Could you check a few things on this model? Use its own coordinates, in mm. Coordinates: 2 decimals unless noted, no trailing zeros. Loops run counter-clockwise (first coordinate to the right, second up) from the corner with the lowest first, then second, coordinate; pieces in that order, holes last. Notation, with made-up numbers: M 80,48.5 L 131,48.5 A16 cw 131,64.5 Z; hole C -8.5,66 d9. An arc over 180 degrees is marked long. Use one line per item in the form item = value. Start each with the question number.
```python
from build123d import *

# Parameters (mm, degrees)
SKETCH_1_W          = 90
SKETCH_1_H          = 110
EXTRUDE_1_DEPTH     = 6
SKETCH_2_R          = 4.5
SKETCH_2_R_2        = 10.1
CUT_EXTRUDE_1_DEPTH = 16


with BuildPart() as part:
    # 草图1 → 凸台-拉伸1 (new, symmetric)
    with BuildSketch(Plane.XY):
        Rectangle(SKETCH_1_W, SKETCH_1_H)
    extrude(amount=EXTRUDE_1_DEPTH, both=True)

    # 草图2 → 切除-拉伸1 (cut, symmetric)
    with BuildSketch(Plane.XY):
        with Locations((-30, 30)):
            Circle(SKETCH_2_R)
        with Locations((30, 30)):
            Circle(SKETCH_2_R)
        with Locations((0, -10)):
            Circle(SKETCH_2_R_2)
    extrude(amount=CUT_EXTRUDE_1_DEPTH, both=True, mode=Mode.SUBTRACT)


solid = part.part
```
Item 1: I want a section at B-B (x = 30). Write out the boundary of the cut face in (y, z), plus the area to 3 significant figures.
Item 2: I want a section at D-D (y = 30). Write out the boundary of the cut face in (x, z), plus the area to 3 significant figures.
Item 3: Thinking about a two-plate mould opening in Y: for faces 1 (the flat face through (-1, 1, -6)), 2 (the flat face through (-1, 55, 0)), 3 (the cylindrical face through (32.08, 26.01, 0.08)), which applies, pulls with the +Y half, pulls with the -Y half, needs draft (parallel to the pull), parting line crosses it, or undercut?
Item 4: Please list where these lines run through material, in increasing order: line 1 along X through (y, z) = (30, 1.75); line 2 along Y through (x, z) = (-30, 2); line 3 along X through (y, z) = (32.5, 4).
Item 5: I want a section at C-C (z = -3.25). Write out the boundary of the cut face in (x, y).
Item 6: I want a section at A-A (y = -10). Write out the boundary of the cut face in (x, z).
Worked answers:
q1.outline = M -55,-6 L 25.5,-6 L 25.5,6 L -55,6 Z; M 34.5,-6 L 55,-6 L 55,6 L 34.5,6 Z
q1.area = 1,210 mm²
q2.outline = M -45,-6 L -34.5,-6 L -34.5,6 L -45,6 Z; M -25.5,-6 L 25.5,-6 L 25.5,6 L -25.5,6 Z; M 34.5,-6 L 45,-6 L 45,6 L 34.5,6 Z
q2.area = 864 mm²
q3.face_1 = needs draft
q3.face_2 = pulls with the +Y half
q3.face_3 = undercut
q4.line_1 = -45 to -34.5, -25.5 to 25.5, 34.5 to 45
q4.line_2 = -55 to 25.5, 34.5 to 55
q4.line_3 = -45 to -33.74, -26.26 to 26.26, 33.74 to 45
q5.outline = M -45,-55 L 45,-55 L 45,55 L -45,55 Z; hole C -30,30 d9; hole C 0,-10 d20.2; hole C 30,30 d9
q6.outline = M -45,-6 L -10.1,-6 L -10.1,6 L -45,6 Z; M 10.1,-6 L 45,-6 L 45,6 L 10.1,6 Z
